```python
from build123d import *

# Parameters (mm, degrees)
BASE_BLOCK_SKETCH_W         = 100
BASE_BLOCK_SKETCH_H         = 100
BASE_BLOCK_100X100X30_DEPTH = 30
FLANGE_PLATE_DEPTH          = 10
CENTRE_BOSS_DEPTH           = 10
BOSS_HOLES_SKETCH_R         = 5
BOSS_HOLES_4X_10_DEPTH      = 10
FLANGE_HOLES_SKETCH_R       = 5
FLANGE_HOLES_4X_10_DEPTH    = 10


with BuildPart() as part:
    # Base Block Sketch → Base Block 100x100x30 (new body)
    with BuildSketch(Plane.XY):
        with Locations((50, -50)):
            Rectangle(BASE_BLOCK_SKETCH_W, BASE_BLOCK_SKETCH_H)
    extrude(amount=BASE_BLOCK_100X100X30_DEPTH)

    # Flange Plate Sketch → Flange Plate (add)
    with BuildSketch(Plane.XY.offset(30)):
        with BuildLine():
            Line((5, -65), (5, -80))
            ThreePointArc((5, -80), (9.393398282, -90.606601718), (20, -95))
            Line((20, -95), (35, -95))
            ThreePointArc((35, -95), (50, -80), (65, -95))
            Line((65, -95), (80, -95))
            ThreePointArc((80, -95), (90.606601718, -90.606601718), (95, -80))
            Line((95, -80), (95, -65))
            ThreePointArc((95, -65), (80, -50), (95, -35))
            Line((95, -35), (95, -20))
            ThreePointArc((95, -20), (90.606601718, -9.393398282), (80, -5))
            Line((80, -5), (65, -5))
            ThreePointArc((65, -5), (50, -20), (35, -5))
            Line((35, -5), (20, -5))
            ThreePointArc((20, -5), (9.393398282, -9.393398282), (5, -20))
            Line((5, -20), (5, -35))
            ThreePointArc((5, -35), (20, -50), (5, -65))
        make_face()
    extrude(amount=FLANGE_PLATE_DEPTH)

    # Centre Boss Sketch → Centre Boss (add)
    with BuildSketch(Plane.XY.offset(40)):
        with BuildLine():
            Line((25, -40), (25, -60))
            ThreePointArc((25, -60), (29.393398282, -70.606601718), (40, -75))
            Line((40, -75), (60, -75))
            ThreePointArc((60, -75), (70.606601718, -70.606601718), (75, -60))
            Line((75, -60), (75, -40))
            ThreePointArc((75, -40), (70.606601718, -29.393398282), (60, -25))
            Line((60, -25), (40, -25))
            ThreePointArc((40, -25), (29.393398282, -29.393398282), (25, -40))
        make_face()
    extrude(amount=CENTRE_BOSS_DEPTH)

    # Boss Holes Sketch → Boss Holes 4xØ10 (cut)
    with BuildSketch(Plane.XY.offset(50)):
        with Locations((40, -40)):
            Circle(BOSS_HOLES_SKETCH_R)
        with Locations((60, -40)):
            Circle(BOSS_HOLES_SKETCH_R)
        with Locations((60, -60)):
            Circle(BOSS_HOLES_SKETCH_R)
        with Locations((40, -60)):
            Circle(BOSS_HOLES_SKETCH_R)
    extrude(amount=-BOSS_HOLES_4X_10_DEPTH, mode=Mode.SUBTRACT)

    # Flange Holes Sketch → Flange Holes 4xØ10 (cut)
    with BuildSketch(Plane.XY.offset(40)):
        with Locations((20, -20)):
            Circle(FLANGE_HOLES_SKETCH_R)
        with Locations((80, -20)):
            Circle(FLANGE_HOLES_SKETCH_R)
        with Locations((80, -80)):
            Circle(FLANGE_HOLES_SKETCH_R)
        with Locations((20, -80)):
            Circle(FLANGE_HOLES_SKETCH_R)
    extrude(amount=-FLANGE_HOLES_4X_10_DEPTH, mode=Mode.SUBTRACT)


solid = part.part
```
The listing builds one solid part. Answer for the finished solid, in the listing's coordinates (mm). A direction names the side the tool comes from. Give positions to 0.01 mm unless a question says otherwise; leave off trailing zeros. Order: outer loops, then holes, each group sorted by start corner. A loop starts at its lowest first (then second) coordinate and runs counter-clockwise, first axis right, second up.
1) Consider line 1 along Y through (x, z) = (60, 45); line 2 along Y through (x, z) = (39, 44.5); line 3 along Z through (x, y) = (57, -95.5). Determine where each line is inside the solid, lowest interval first.
Reported:
line 1: y = -75 to -65, -55 to -45, -35 to -25
line 2: y = -74.97 to -64.9, -55.1 to -44.9, -35.1 to -25.03
line 3: z = 0 to 30
2) Given P1, Ø5, axis at x = 74, z = 36, coming from the -Y side; P2, Ø3, axis at x = 75, z = 36, coming from the +Y side; P3, Ø4, axis at x = 83.5, y = -74.5, coming from the +Z side, each flat-ended and moving along its own axis, determine where each tip first touches the part or whether it passes through.
Reported:
P1: stops at y = -95
P2: stops at y = -5
P3: stops at z = 40
3) Find section B-B on x = 13. Write down the section's boundary in (y, z), then the cut area to 3 significant figures.
Reported:
outline: (-100, 0) - (0, 0) - (0, 30) - (-6.73, 30) - (-6.73, 40) - (-37.31, 40) - (-37.31, 30) - (-62.69, 30) - (-62.69, 40) - (-93.27, 40) - (-93.27, 30) - (-100, 30) - close
area: 3,610 mm2
4) Determine the mould class of faces 1 (the face through (40, -60, 40)), 2 (the face through (59.349, -55.043, 45.07)), 3 (the face through (70.72, -29.51, 44.93)), 4 (the face through (9.51, -9.28, 34.93)) for opening direction X: pulls with the +X half, pulls with the -X half, needs draft (parallel to the pull), parting line crosses it, or undercut.
Reported:
face 1: undercut
face 2: undercut
face 3: pulls with the +X half
face 4: pulls with the -X half
5) For faces 5 (the face through (50, -25, 45)), 6 (the face through (75, -50, 45)), 7 (the face through (29.28, -70.49, 44.93)), 8 (the face through (50, -20, 35)), determine the directions among +Z, -Z, +X, -X, +Y, -Y from which every point of the face is accessible in a straight line to the end or side of a thin tool.
Reported:
face 5: +Z, +X, -X, +Y
face 6: +Z, +X, +Y, -Y
face 7: +Z, -X, -Y
face 8: +Z, +Y
6) Find section A-A on y = -50. Write down the section's boundary in (x, z), then the cut area to 3 significant figures.
Reported:
outline: (0, 0) - (100, 0) - (100, 30) - (80, 30) - (80, 40) - (75, 40) - (75, 50) - (25, 50) - (25, 40) - (20, 40) - (20, 30) - (0, 30) - close
area: 4,100 mm2
